```python
from build123d import *

# Parameters (mm, degrees)
SKETCH1_R           = 30.5
SKETCH1_R_2         = 26.25
BOSS_EXTRUDE1_DEPTH = 1
CHAMFER1_SIZE       = 1.5
CHAMFER1_SIZE2      = 1
BOSS_EXTRUDE2_START = -2
BOSS_EXTRUDE2_DEPTH = 2
CIRPATTERN2_COUNT   = 8


with BuildPart() as part:
    # Sketch1 → Boss-Extrude1 (new, symmetric)
    with BuildSketch(Plane.XY):
        Circle(SKETCH1_R)
        Circle(SKETCH1_R_2, mode=Mode.SUBTRACT)
    extrude(amount=BOSS_EXTRUDE1_DEPTH, both=True)

    # Chamfer1
    chamfer1_edges = [part.edges().sort_by_distance(p)[0] for p in [
        (-30.5, 0, -1),
    ]]
    chamfer1_side = [part.faces().sort_by_distance(p)[0] for p in [
        (-29.637329727, 0, -1),
    ]]
    chamfer(chamfer1_edges, length=CHAMFER1_SIZE, length2=CHAMFER1_SIZE2, reference=chamfer1_side[0])

    # Sketch4 → Boss-Extrude2 (add)
    with BuildSketch(Plane.XY.offset(1).offset(BOSS_EXTRUDE2_START)):
        with BuildLine():
            Line((-3, 25), (-3, 26.078007976))
            ThreePointArc((-3, 26.078007976), (0, 26.25), (3, 26.078007976))
            Line((3, 26.078007976), (3, 25))
            ThreePointArc((3, 25), (0, 22), (-3, 25))
        make_face()
    boss_extrude2 = extrude(amount=BOSS_EXTRUDE2_DEPTH)

    # Sketch5 → CSK for M2.5 Countersunk Flat Head Screw2 (revolve, cut)
    with BuildSketch(Plane(origin=(0, 25, 1), x_dir=(0, -1, 0), z_dir=(1, 0, 0))):
        Polygon((0, 0), (0, 2), (1.45, 2), (1.45, 1.3), (2.75, 0), align=None)
    csk_for_m2_5_countersunk_flat_head_screw = revolve(axis=Axis((0, 25, 7.35), (0, 0, -1)), mode=Mode.SUBTRACT)

    # CirPattern2: Boss-Extrude2, CSK for M2.5 Countersunk Flat Head Screw2 ×8 about axis
    cirpattern2_axis = Axis((0, 0, 0), (0, 0, 1))
    add([boss_extrude2.rotate(cirpattern2_axis, i * 360 / CIRPATTERN2_COUNT) for i in range(1, CIRPATTERN2_COUNT)])
    add([csk_for_m2_5_countersunk_flat_head_screw.rotate(cirpattern2_axis, i * 360 / CIRPATTERN2_COUNT) for i in range(1, CIRPATTERN2_COUNT)], mode=Mode.SUBTRACT)


solid = part.part
```
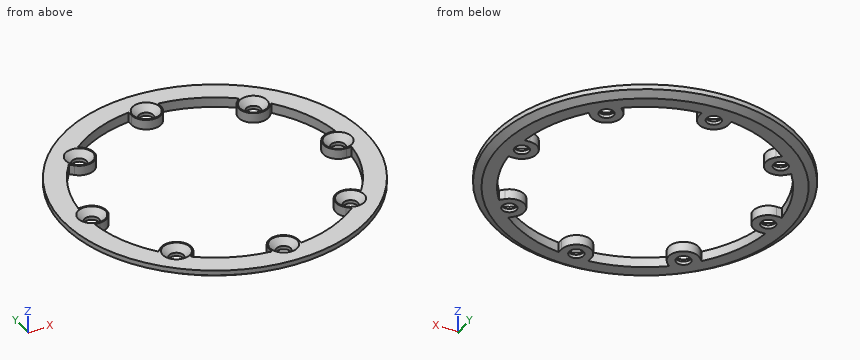
For this review, take the finished solid that the model builds, in its own axes (mm). Give positions to 0.01 mm unless a question says otherwise; leave off trailing zeros. Write each loop counter-clockwise with the first axis right and the second up, starting at its lowest first coordinate (ties: lowest second). Pieces come first, ordered by that corner, then holes.
Item 1: Insertion check: P1, Ø2.5, axis at x = 0, y = 25, coming from the +Z side; P2, Ø0.9, axis at x = 25.5, z = 0, coming from the -Y side; P3, Ø0.5, axis at y = 25.5, z = 0.5, coming from the -X side; P4, Ø4.5, axis at x = 17.68, y = -17.68, coming from the +Z side. Each pin has a flat end and moves straight along its axis. Give the tip position at first contact, or say it passes through.
Item 2: Wall thickness on probe 1 along Y at (x, z) = (15.5, -0.9); probe 2 along X at (y, z) = (-19, -0.85); probe 3 along Y at (x, z) = (0.5, -0.15): over which ranges is each line inside the solid? List them lowest first.
Item 3: Take a section at A-A (x = 0). Give the boundary of the cut face in (y, z), and give its area (3 significant figures).
Item 4: Take a section at C-C (z = 0.3). Give the number of separate pieces and of enclosed holes in the cut face, and give its area (3 significant figures).
Established:
1. P1: passes through
1. P2: stops at y = -17.4
1. P3: stops at x = -17.11
1. P4: stops at z = 0.5
2. probe 1: y = -24.69 to -21.19, -19.74 to -15.61, 15.61 to 19.74, 21.19 to 24.69
2. probe 2: x = -22.21 to -18.27, -17.08 to -14.98, 14.98 to 17.08, 18.27 to 22.21
2. probe 3: y = -30.27 to -26.52, -23.48 to -22.04, 22.04 to 23.48, 26.52 to 30.27
3. outline: (-30.5, 0) - (-29, -1) - (-26.45, -1) - (-26.45, -0.3) - (-27.75, 1) - (-30.5, 1) - close; (-23.55, -1) - (-22, -1) - (-22, 1) - (-22.25, 1) - (-23.55, -0.3) - close; (22, -1) - (23.55, -1) - (23.55, -0.3) - (22.25, 1) - (22, 1) - close; (26.45, -1) - (29, -1) - (30.5, 0) - (30.5, 1) - (27.75, 1) - (26.45, -0.3) - close
3. area: 17.5 mm2
4. separate pieces: 1
4. enclosed holes: 9
4. area: 822 mm2
